Could you check a few things on this model? Use its own coordinates, in mm. Face numbers are marked on the shaded views. A direction names the side the tool comes from. Coordinates: 2 decimals unless noted, no trailing zeros. Write each loop counter-clockwise with the first axis right and the second up, starting at its lowest first coordinate (ties: lowest second). Pieces come first, ordered by that corner, then holes.
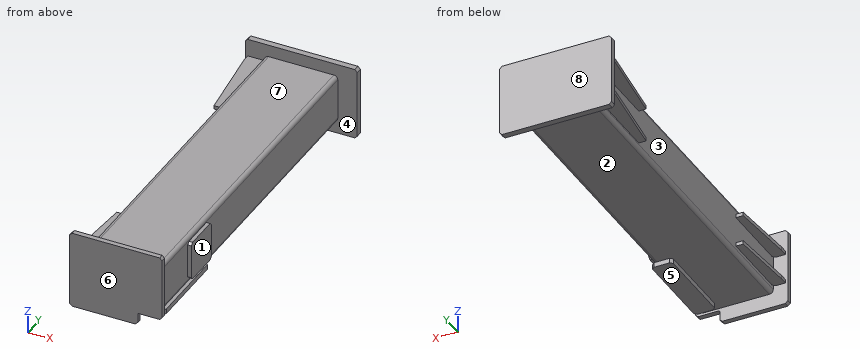
```python
from build123d import *

# Parameters (mm, degrees)
BOSS_EXTRUDE1_DEPTH  = 20
BOSS_EXTRUDE2_DEPTH  = 1431
BOSS_EXTRUDE3_DEPTH  = 25
BOSS_EXTRUDE4_START  = -22.5
BOSS_EXTRUDE4_DEPTH  = 15
BOSS_EXTRUDE5_DEPTH  = 15
BOSS_EXTRUDE9_START  = -30
BOSS_EXTRUDE9_DEPTH  = 15
BOSS_EXTRUDE10_DEPTH = 20


with BuildPart() as part:
    # Sketch1 → Boss-Extrude1 (new body)
    with BuildSketch(Plane(origin=(0, 0, 0), x_dir=(1, 0, 0), z_dir=(0, 1, 0))):
        with BuildLine():
            Line((-3.496816057, 9.368686005), (-3.496816057, 309.368686005))
            Line((-3.496816057, 309.368686005), (6.503183943, 319.368686005))
            Line((6.503183943, 319.368686005), (141.657748152, 319.368686005))
            Line((141.657748152, 319.368686005), (266.503183943, 319.368686005))
            Line((266.503183943, 319.368686005), (276.503183943, 309.368686005))
            Line((276.503183943, 309.368686005), (276.503183943, 274.368686005))
            ThreePointArc((276.503183943, 274.368686005), (277.967650037, 270.833152099), (281.503183943, 269.368686005))
            Line((281.503183943, 269.368686005), (366.503183943, 269.368686005))
            Line((366.503183943, 269.368686005), (376.503183943, 259.368686005))
            Line((376.503183943, 259.368686005), (376.503183943, 9.368686005))
            Line((376.503183943, 9.368686005), (366.503183943, -0.631313995))
            Line((366.503183943, -0.631313995), (6.503183943, -0.631313995))
            Line((6.503183943, -0.631313995), (-3.496816057, 9.368686005))
        make_face()
    extrude(amount=BOSS_EXTRUDE1_DEPTH)

    # Sketch2 → Boss-Extrude2 (add)
    with BuildSketch(Plane(origin=(0, 20, 0), x_dir=(1, 0, 0), z_dir=(0, 1, 0))):
        with BuildLine():
            Line((72.503183943, 259.368686005), (340.503183943, 259.368686005))
            ThreePointArc((340.503183943, 259.368686005), (351.816892442, 254.682394504), (356.503183943, 243.368686005))
            Line((356.503183943, 243.368686005), (356.503183943, 75.368686005))
            ThreePointArc((356.503183943, 75.368686005), (351.816892442, 64.054977506), (340.503183943, 59.368686005))
            Line((340.503183943, 59.368686005), (72.503183943, 59.368686005))
            ThreePointArc((72.503183943, 59.368686005), (61.189475444, 64.054977506), (56.503183943, 75.368686005))
            Line((56.503183943, 75.368686005), (56.503183943, 243.368686005))
            ThreePointArc((56.503183943, 243.368686005), (61.189475444, 254.682394504), (72.503183943, 259.368686005))
        make_face()
        with BuildLine():
            Line((72.503183943, 251.368686005), (340.503183943, 251.368686005))
            ThreePointArc((340.503183943, 251.368686005), (346.160038192, 249.025540255), (348.503183943, 243.368686005))
            Line((348.503183943, 243.368686005), (348.503183943, 75.368686005))
            ThreePointArc((348.503183943, 75.368686005), (346.160038192, 69.711831756), (340.503183943, 67.368686005))
            Line((340.503183943, 67.368686005), (72.503183943, 67.368686005))
            ThreePointArc((72.503183943, 67.368686005), (66.846329693, 69.711831756), (64.503183943, 75.368686005))
            Line((64.503183943, 75.368686005), (64.503183943, 243.368686005))
            ThreePointArc((64.503183943, 243.368686005), (66.846329693, 249.025540255), (72.503183943, 251.368686005))
        make_face(mode=Mode.SUBTRACT)
    extrude(amount=BOSS_EXTRUDE2_DEPTH)

    # Sketch3 → Boss-Extrude3 (add)
    with BuildSketch(Plane(origin=(0, 1451, 0), x_dir=(1, 0, 0), z_dir=(0, 1, 0))):
        Polygon((-13.496816057, 309.368686005), (426.503183943, 309.368686005), (436.503183943, 299.368686005), (436.503183943, 19.368686005), (426.503183943, 9.368686005), (-13.496816057, 9.368686005), (-23.496816057, 19.368686005), (-23.496816057, 299.368686005), align=None)
    extrude(amount=BOSS_EXTRUDE3_DEPTH)

    # Sketch4 → Boss-Extrude4 (add)
    with BuildSketch(Plane.XY.offset(-59.368686005).offset(BOSS_EXTRUDE4_START)):
        Polygon((-13.496816057, 1451), (46.503183943, 1451), (56.503183943, 1441), (56.503183943, 1101), (26.503183943, 1101), (-13.496816057, 1421), align=None)
    boss_extrude4 = extrude(amount=-BOSS_EXTRUDE4_DEPTH)

    # Mirror1: Boss-Extrude4 across plane
    add(boss_extrude4.mirror(Plane.XY.offset(-159.368686005)))

    # Sketch5 → Boss-Extrude5 (add)
    with BuildSketch(Plane(origin=(356.503183943, 0, 0), x_dir=(0, 0, -1), z_dir=(1, 0, 0))):
        Polygon((89.368686005, 405), (229.368686005, 405), (239.368686005, 395), (239.368686005, 255), (229.368686005, 245), (89.368686005, 245), (79.368686005, 255), (79.368686005, 395), align=None)
    extrude(amount=BOSS_EXTRUDE5_DEPTH)

    # Sketch9 → Boss-Extrude9 (add)
    with BuildSketch(Plane.XY.offset(-59.368686005).offset(BOSS_EXTRUDE9_START)):
        Polygon((56.503183943, 30), (56.503183943, 320), (26.503183943, 320), (6.503183943, 50), (6.503183943, 20), (46.503183943, 20), align=None)
    boss_extrude9 = extrude(amount=-BOSS_EXTRUDE9_DEPTH)

    # Mirror2: Boss-Extrude9 across plane
    add(boss_extrude9.mirror(Plane.XY.offset(-159.368686005)))

    # Sketch10 → Boss-Extrude10 (add)
    with BuildSketch(Plane(origin=(0, 0, -259.368686005), x_dir=(-1, 0, 0), z_dir=(0, 0, -1))):
        Polygon((-353.503183943, 399), (-288.503183943, 399), (-278.503183943, 389), (-278.503183943, 59), (-288.503183943, 49), (-353.503183943, 49), (-363.503183943, 59), (-363.503183943, 389), align=None)
    extrude(amount=BOSS_EXTRUDE10_DEPTH)


solid = part.part
```
Item 1: If we mould it in two halves opening along Z, with no side actions, what happens to the marked faces 1, 2 and 3? For each: released by +Z, released by -Z, zero draft, split by the parting line, or undercut.
Item 2: I want a section at B-B, the plane z = -177. List the corners of the cut face in (x, y) for me.
Item 3: I want a section at A-A, the plane y = 823. List the corners of the cut face in (x, z) for me.
Item 4: I want a section at C-C, the plane x = 187. List the corners of the cut face in (y, z) for me.
Item 5: Which directions (+Z, -Z, +X, -X, +Y, -Y) give clear straight access to the entire face, cutting with the end or side of a thin tool? Please do the marked faces 4, 5, 6, 7 and 8.
Item 6: Will these pins go through, and if not, where does the flat tip stop? pin 1 Ø4 at (y, z) = (753, -76) entering from -X; pin 2 Ø12 at (x, y) = (104, 528) entering from +Z; pin 3 Ø4.5 at (y, z) = (38, -97.5) entering from -X; pin 4 Ø12 at (y, z) = (1154, -49.5) entering from -X.
Item 7: If I drill on line 1 along Y through (x, z) = (35, -21); line 2 along X through (y, z) = (104, -182.5); line 3 along Y through (x, z) = (349, -272), over which ranges is the centre line in solid material (lowest first)?
Taken from the geometry:
1. face 1: zero draft
1. face 2: released by -Z
1. face 3: undercut
2. outline: (-23.5, 1451) - (56.5, 1451) - (56.5, 20) - (-3.5, 20) - (-3.5, 0) - (376.5, 0) - (376.5, 20) - (356.5, 20) - (356.5, 245) - (371.5, 245) - (371.5, 405) - (356.5, 405) - (356.5, 1451) - (436.5, 1451) - (436.5, 1476) - (-23.5, 1476) - close; hole (64.5, 20) - (348.5, 20) - (348.5, 1451) - (64.5, 1451) - close
3. outline: (56.5, -243.37) arc R16 ccw to (72.5, -259.37) - (340.5, -259.37) arc R16 ccw to (356.5, -243.37) - (356.5, -75.37) arc R16 ccw to (340.5, -59.37) - (72.5, -59.37) arc R16 ccw to (56.5, -75.37) - close; hole (64.5, -243.37) arc R8 ccw to (72.5, -251.37) - (340.5, -251.37) arc R8 ccw to (348.5, -243.37) - (348.5, -75.37) arc R8 ccw to (340.5, -67.37) - (72.5, -67.37) arc R8 ccw to (64.5, -75.37) - close
4. outline: (0, -319.37) - (20, -319.37) - (20, -259.37) - (1451, -259.37) - (1451, -309.37) - (1476, -309.37) - (1476, -9.37) - (1451, -9.37) - (1451, -59.37) - (20, -59.37) - (20, 0.63) - (0, 0.63) - close; hole (20, -251.37) - (1451, -251.37) - (1451, -67.37) - (20, -67.37) - close
5. face 4: none
5. face 5: -Z, +X, -X, -Y
5. face 6: +Z, -Z, +X, -X, -Y
5. face 7: +Z, +X, -X
5. face 8: +Z, -Z, +X, -X, +Y
6. pin 1: stops at x = 56.5
6. pin 2: stops at z = -59.37
6. pin 3: stops at x = 6.5
6. pin 4: passes through
7. line 1: y = 0 to 20, 1451 to 1476
7. line 2: x = 56.5 to 64.5, 348.5 to 356.5
7. line 3: y = 49 to 399, 1451 to 1476
